from build123d import *

# Parameters (mm, degrees)
BOSS_EXTRUDE1_DEPTH   = 12
SKETCH2_R             = 13
CUT_EXTRUDE1_DEPTH    = 126.427269762
M8_TAPPED_HOLE1_D     = 6.8
M8_TAPPED_HOLE1_DEPTH = 19.75
M8_TAPPED_HOLE1_TIP   = 2.042926105
M5_TAPPED_HOLE1_D     = 4.2
M5_TAPPED_HOLE1_DEPTH = 12.4
M5_TAPPED_HOLE1_TIP   = 1.2618073
M5_TAPPED_HOLE2_D     = 4.2
M5_TAPPED_HOLE2_DEPTH = 12.4
M5_TAPPED_HOLE2_TIP   = 1.2618073
CHAMFER1_SIZE         = 3
SKETCH11_R            = 1.5
CUT_EXTRUDE2_DEPTH    = 126.427269762


with BuildPart() as part:
    # Sketch1 → Boss-Extrude1 (new body)
    with BuildSketch(Plane(origin=(0, 0, 0), x_dir=(0, 0, -1), z_dir=(1, 0, 0))):
        Polygon((0, 0), (102, 0), (102, 60), (32, 60), (32, 72), (0, 72), align=None)
    extrude(amount=BOSS_EXTRUDE1_DEPTH)

    # Sketch2 → Cut-Extrude1 (cut, through all)
    with BuildSketch(Plane(origin=(12, 0, 0), x_dir=(0, 0, -1), z_dir=(1, 0, 0))):
        with Locations((46.5, 27.5)):
            Circle(SKETCH2_R)
    extrude(amount=-CUT_EXTRUDE1_DEPTH, mode=Mode.SUBTRACT)

    # M8 Tapped Hole1
    with Locations(Plane.ZY):
        with Locations((-77.5, 45.5), (-77.5, 9.5), (-15.5, 9.5), (-15.5, 45.5)):
            Hole(M8_TAPPED_HOLE1_D / 2, depth=M8_TAPPED_HOLE1_DEPTH)
            with Locations((0, 0, -(M8_TAPPED_HOLE1_DEPTH + M8_TAPPED_HOLE1_TIP / 2))):  # 118° drill point
                Cone(0, M8_TAPPED_HOLE1_D / 2, M8_TAPPED_HOLE1_TIP, mode=Mode.SUBTRACT)

    # M5 Tapped Hole1
    with Locations(Plane(origin=(12, 0, 0), x_dir=(0, 0, -1), z_dir=(1, 0, 0))):
        with Locations((67, 35), (67, 15)):
            Hole(M5_TAPPED_HOLE1_D / 2, depth=M5_TAPPED_HOLE1_DEPTH)
            with Locations((0, 0, -(M5_TAPPED_HOLE1_DEPTH + M5_TAPPED_HOLE1_TIP / 2))):  # 118° drill point
                Cone(0, M5_TAPPED_HOLE1_D / 2, M5_TAPPED_HOLE1_TIP, mode=Mode.SUBTRACT)

    # M5 Tapped Hole2
    with Locations(Plane(origin=(0, 60, 0), x_dir=(1, 0, 0), z_dir=(0, 1, 0))):
        with Locations((6, 42), (6, 92)):
            Hole(M5_TAPPED_HOLE2_D / 2, depth=M5_TAPPED_HOLE2_DEPTH)
            with Locations((0, 0, -(M5_TAPPED_HOLE2_DEPTH + M5_TAPPED_HOLE2_TIP / 2))):  # 118° drill point
                Cone(0, M5_TAPPED_HOLE2_D / 2, M5_TAPPED_HOLE2_TIP, mode=Mode.SUBTRACT)

    # Chamfer1
    chamfer1_edges = [part.edges().sort_by_distance(p)[0] for p in [
        (6, 72, 0),
        (6, 0, -102),
        (6, 0, 0),
    ]]
    chamfer(chamfer1_edges, length=CHAMFER1_SIZE)

    # Sketch11 → Cut-Extrude2 (cut, through all)
    with BuildSketch(Plane(origin=(12, 0, 0), x_dir=(0, 0, -1), z_dir=(1, 0, 0))):
        with Locations((32, 60)):
            Circle(SKETCH11_R)
    extrude(amount=-CUT_EXTRUDE2_DEPTH, mode=Mode.SUBTRACT)


solid = part.part
Work out the finished part from the listing and answer in its coordinate system (mm). A direction names the side the tool comes from. Round coordinates to 2 decimals unless told otherwise and drop trailing zeros. Loops run counter-clockwise (first coordinate to the right, second up) from the corner with the lowest first, then second, coordinate; pieces in that order, holes last. Notation, with made-up numbers: (30, 37) - (82, 37) arc R23 cw to (82, 52) - close; hole circle Ø7 at (-3, 50.25). An arc over 180 degrees is marked (long way). One line per item, written item: value.
Q1. Find section B-B on y = 52.5. Give the vertices of the cut face in (x, z), and give its area (3 significant figures).
Check values:
outline: (0, -102) - (12, -102) - (12, 0) - (0, 0) - close; hole circle Ø4.2 at (6, -92); hole circle Ø4.2 at (6, -42)
area: 1,200 mm2
Q2. Find section D-D on y = 35. Give the vertices of the cut face in (x, z), and give its area (3 significant figures).
Check values:
outline: (0, -102) - (12, -102) - (12, -69.1) - (0, -69.1) - close; (0, -64.9) - (12, -64.9) - (12, -57.12) - (0, -57.12) - close; (0, -35.88) - (12, -35.88) - (12, 0) - (0, 0) - close
area: 919 mm2
Q3. For faces 4 (the cylindrical face through (6.08, 48.87, -77.06)), 5 (the flat face through (6, 67, -32)), determine the directions among +Z, -Z, +X, -X, +Y, -Y from which every point of the face is accessible in a straight line to the end or side of a thin tool.
Check values:
face 4: +X, -X
face 5: -Z, +X, -X, +Y
Q4. The mould has two halves that part along Y. Classify faces 1 (the cylindrical face through (7.666, 53.713, -90.722)), 2 (the conical face through (5.73, 46.56, -42.25)), 3 (the cylindrical face through (5.916, 33.137, -66.031)): +Y half, -Y half, draft (parallel to the pull), parting line (faces both ways), or undercut.
Check values:
face 1: draft
face 2: +Y half
face 3: undercut
Q5. Find section A-A on z = -77.5. Give the vertices of the cut face in (x, y), and give its area (3 significant figures).
Check values:
outline: (0, 0) - (12, 0) - (12, 6.1) - (0, 6.1) - close; (0, 12.9) - (12, 12.9) - (12, 42.1) - (0, 42.1) - close; (0, 48.9) - (12, 48.9) - (12, 60) - (0, 60) - close
area: 557 mm2
Q6. This flat-tipped pin is pushed along its axis until it touches: pin 1 Ø4 at (y, z) = (15, -67) entering from +X. Where does it stop, or does it pass through?
Check values:
pin 1: through
Q7. Straight lines are drawn through the part: probe 1 along Y at (x, z) = (6, -67); probe 2 along Z at (x, y) = (6, 53.25); probe 3 along X at (y, z) = (55, -42). For each, find the intervals that lie inside material, in ascending order.
Check values:
probe 1: 0 to 12.9, 17.1 to 32.9, 37.1 to 60
probe 2: -102 to -94.1, -89.9 to -44.1, -39.9 to 0
probe 3: 0 to 3.9, 8.1 to 12
Q8. Find section C-C on y = 18.5. Give the vertices of the cut face in (x, z).
Check values:
outline: (0, -102) - (12, -102) - (12, -55.88) - (0, -55.88) - close; (0, -37.12) - (12, -37.12) - (12, 0) - (0, 0) - close
